For this review, take the finished solid that the model builds, in its own axes (mm). Face numbers are marked on the shaded views. A direction names the side the tool comes from. Round coordinates to 2 decimals unless told otherwise and drop trailing zeros. Loops run counter-clockwise (first coordinate to the right, second up) from the corner with the lowest first, then second, coordinate; pieces in that order, holes last.
1) Tool access review of the marked faces 1, 2 and 3: name each direction out of +Z, -Z, +X, -X, +Y, -Y from which nothing blocks a thin tool from reaching the whole face with its end or side.
2) Take a section at A-A (z = 0). State the section outline as (x, y) points, then the cut area to 3 significant figures.
3) Insertion check: pin 1 (6 mm diameter, centred on y = 6.5, z = -4, fed in from +X); pin 2 (5 mm diameter, centred on x = -44.5, y = 8, fed in from -Z); pin 3 (6 mm diameter, centred on x = -57, z = -8, fed in from +Y); pin 4 (1.5 mm diameter, centred on x = -54.5, z = -7, fed in from +Y). Each pin has a flat end and moves straight along its axis. Give the tip position at first contact, or say it passes through.
4) Take a section at C-C (x = -16.5). State the section outline as (y, z) points.
5) Wall thickness on L1, parallel to X at y = -8, z = -5.5; L2, parallel to Z at x = -60.5, y = 0.5; L3, parallel to Z at x = -49.5, y = 2: over which ranges is each line inside the solid? List them lowest first.
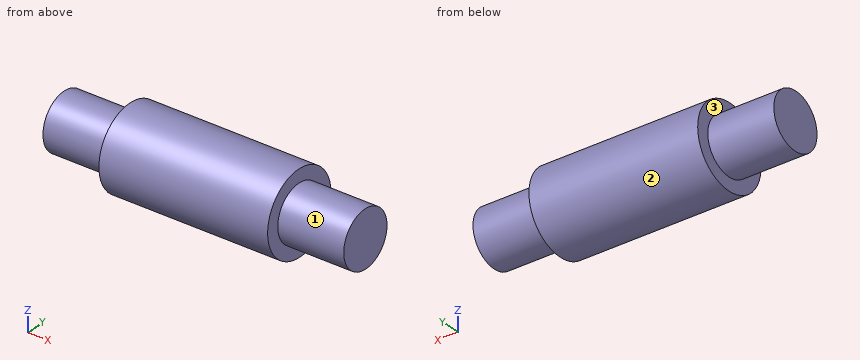
```python
from build123d import *


with BuildPart() as part:
    # Spacer Profile Sketch → Spacer Body Revolve (revolve)
    with BuildSketch(Plane.XY):
        Polygon((-82, 0), (-82, 7.5), (-64, 7.5), (-64, 11), (-18, 11), (-18, 7.5), (0, 7.5), (0, 0), align=None)
    revolve(axis=Axis((0, 0, 0), (-1, 0, 0)))


solid = part.part
```
Response:
1. face 1: +X
1. face 2: +X, -X
1. face 3: -X
2. outline: (-82, -7.5) - (-64, -7.5) - (-64, -11) - (-18, -11) - (-18, -7.5) - (0, -7.5) - (0, 7.5) - (-18, 7.5) - (-18, 11) - (-64, 11) - (-64, 7.5) - (-82, 7.5) - close
2. area: 1,550 mm2
3. pin 1: stops at x = 0
3. pin 2: stops at z = -9.53
3. pin 3: stops at y = 9.8
3. pin 4: stops at y = 9.05
4. outline: circle Ø15 at (0, 0)
5. L1: x = -64 to -18
5. L2: z = -10.99 to 10.99
5. L3: z = -10.82 to 10.82
